```python
from build123d import *

# Parameters (mm, degrees)
SKETCH_1_R          = 72.5
EXTRUDE_1_DEPTH     = 25
SKETCH_2_R          = 7
CUT_EXTRUDE_1_DEPTH = 106.534354596
CUT_EXTRUDE_2_DEPTH = 15
CHAMFER_1_SIZE      = 1
CHAMFER_2_SIZE      = 1


with BuildPart() as part:
    # 草图1 → 凸台-拉伸1 (new body)
    with BuildSketch(Plane.XY):
        Circle(SKETCH_1_R)
    extrude(amount=EXTRUDE_1_DEPTH)

    # 草图2 → 切除-拉伸1 (cut, through all)
    with BuildSketch(Plane.XY.offset(25)):
        with Locations((0, 60)):
            Circle(SKETCH_2_R)
        with Locations((60, 0)):
            Circle(SKETCH_2_R)
        with Locations((0, -60)):
            Circle(SKETCH_2_R)
        with Locations((-60, 0)):
            Circle(SKETCH_2_R)
    extrude(amount=-CUT_EXTRUDE_1_DEPTH, mode=Mode.SUBTRACT)

    # 草图3 → 切除-拉伸2 (cut)
    with BuildSketch(Plane(origin=(0, 0, 0), x_dir=(-1, 0, 0), z_dir=(0, 0, -1))):
        with BuildLine():
            Line((-32.5, 36), (32.5, 36))
            ThreePointArc((32.5, 36), (48.5, 0), (32.5, -36))
            Line((32.5, -36), (-32.5, -36))
            ThreePointArc((-32.5, -36), (-48.5, 0), (-32.5, 36))
        make_face()
    extrude(amount=-CUT_EXTRUDE_2_DEPTH, mode=Mode.SUBTRACT)

    # 倒角1
    chamfer_1_edges = [part.edges().sort_by_distance(p)[0] for p in [
        (-72.5, 0, 25),
    ]]
    chamfer(chamfer_1_edges, length=CHAMFER_1_SIZE)

    # 倒角2
    chamfer_2_edges = [part.edges().sort_by_distance(p)[0] for p in [
        (48.5, 0, 0),
        (0, -36, 0),
        (-48.5, 0, 0),
        (0, 36, 0),
    ]]
    chamfer(chamfer_2_edges, length=CHAMFER_2_SIZE)


solid = part.part
```
For this review, take the finished solid that the model builds, in its own axes (mm). A direction names the side the tool comes from. Give positions to 0.01 mm unless a question says otherwise; leave off trailing zeros. Order: outer loops, then holes, each group sorted by start corner. A loop starts at its lowest first (then second) coordinate and runs counter-clockwise, first axis right, second up.
1) Wall thickness on line 1 (Z direction, x = -41.5, y = 20.5); line 2 (Y direction, x = 60, z = 17); line 3 (Y direction, x = 43, z = 14): over which ranges is each line inside the solid? List them lowest first.
2) The part is to be moulded in two halves that separate along X. For faces 3 (the face through (-1, -47, 0)), 4 (the face through (66.677, 2.103, 12.675)), 5 (the face through (69.15, 21.78, 11.83)), say which applies: released by +X, released by -X, zero draft, split by the parting line, or undercut.
3) Insertion check: pin 1 (12 mm diameter, centred on x = -38.5, z = 12.5, fed in from -Y); pin 2 (4 mm diameter, centred on x = 13, z = 14.5, fed in from -Y); pin 3 (4 mm diameter, centred on y = -49.5, z = 13, fed in from -X); pin 4 (8.5 mm diameter, centred on x = 0, y = -60, fed in from -Z). Each pin has a flat end and moves straight along its axis. Give the tip position at first contact, or say it passes through.
4) Take a section at A-A (x = 0). Give the boundary of the cut face in (y, z), then the cut area to 3 significant figures.
5) Take a section at C-C (y = 0). Give the boundary of the cut face in (x, z).
6) For faces 1 (the face through (-48.656, 0.575, 0.84)), 2 (the face through (-53.323, 2.103, 12.675)), list the 3-axis set-ups (+Z, -Z, +X, -X, +Y, -Y) from which the entire face can be reached by the end or side of a thin tool; tool diameter is ignored.
7) Take a section at B-B (z = 10). Give the boundary of the cut face in (x, y).
Derived:
1. line 1: z = 15 to 25
1. line 2: y = -40.7 to -7, 7 to 40.7
1. line 3: y = -58.37 to -22.43, 22.43 to 58.37
2. face 3: zero draft
2. face 4: undercut
2. face 5: split by the parting line
3. pin 1: stops at y = -64.81
3. pin 2: stops at y = -71.66
3. pin 3: stops at x = -54.77
3. pin 4: passes through
4. outline: (-72.5, 0) - (-67, 0) - (-67, 25) - (-71.5, 25) - (-72.5, 24) - close; (-53, 0) - (-37, 0) - (-36, 1) - (-36, 15) - (36, 15) - (36, 1) - (37, 0) - (53, 0) - (53, 25) - (-53, 25) - close; (67, 0) - (72.5, 0) - (72.5, 24) - (71.5, 25) - (67, 25) - close
4. area: 1,840 mm2
5. outline: (-72.5, 0) - (-67, 0) - (-67, 25) - (-71.5, 25) - (-72.5, 24) - close; (-53, 0) - (-49.5, 0) - (-48.5, 1) - (-48.5, 15) - (48.5, 15) - (48.5, 1) - (49.5, 0) - (53, 0) - (53, 25) - (-53, 25) - close; (67, 0) - (72.5, 0) - (72.5, 24) - (71.5, 25) - (67, 25) - close
6. face 1: -Z
6. face 2: +Z, -Z
7. outline: circle Ø145 at (0, 0); hole circle Ø14 at (-60, 0); hole (-32.5, -36) - (32.5, -36) arc R48.5 ccw to (32.5, 36) - (-32.5, 36) arc R48.5 ccw to start; hole circle Ø14 at (0, -60); hole circle Ø14 at (0, 60); hole circle Ø14 at (60, 0)
